The listing builds one solid part. Answer for the finished solid, in the listing's coordinates (mm). Coordinates: 2 decimals unless noted, no trailing zeros. Loops run counter-clockwise (first coordinate to the right, second up) from the corner with the lowest first, then second, coordinate; pieces in that order, holes last. Notation, with made-up numbers: (-4.75, 44) - (6.25, 44) arc R15 ccw to (6.25, 52) - close; hole circle Ø6 at (-10.5, 56). An arc over 180 degrees is marked (long way). Return JSON: item names as keys, results as strings. Group by question number.
1. Section C-C (z = 3.4) is taken. Write down the section's boundary in (x, y), and give its area (3 significant figures).
2. Section A-A (y = 13.5) is taken. Write down the section's boundary in (x, z).
3. Each of these flat-tipped pins is pushed along its axis until it touches: P1, Ø3, axis at x = -8.5, y = 6, coming from the -Z side; P2, Ø3.5, axis at x = 13.5, y = 13.5, coming from the +Z side. Where does it stop, or does it pass through?
4. The mould has two halves that part along Y. Classify faces 1 (the face through (-14.71, -11.603, 1.972)), 2 (the face through (0, -16.5, 2)), 3 (the face through (-14.71, 15.397, 1.972)), 4 (the face through (0, 16.5, 2)): pulls with the +Y half, pulls with the -Y half, needs draft (parallel to the pull), parting line crosses it, or undercut.
5. Find the intervals of material crossed by line 1 along Y through (x, z) = (-13.5, 0.95); line 2 along Y through (x, z) = (-12.5, 2.6); line 3 along X through (y, z) = (-13, 1.35), in increasing order.
6. Section B-B (x = -13.5) is taken. Write down the section's boundary in (y, z), and give its area (3 significant figures).
```python
from build123d import *

# Parameters (mm, degrees)
SKETCH1_W                = 35
SKETCH1_H                = 33
BOSS_EXTRUDE1_DEPTH      = 4
M4_CLEARANCE_HOLE1_D     = 4.5
M4_CLEARANCE_HOLE1_DEPTH = 15
M4_CLEARANCE_HOLE1_TIP   = 1.351936393


with BuildPart() as part:
    # Sketch1 → Boss-Extrude1 (new body)
    with BuildSketch(Plane.XY):
        Rectangle(SKETCH1_W, SKETCH1_H)
    extrude(amount=BOSS_EXTRUDE1_DEPTH)

    # M4 Clearance Hole1
    with Locations(Plane.XY.offset(4)):
        with Locations((13.5, 13.5), (-13.5, 13.5), (-13.5, -13.5), (13.5, -13.5)):
            Hole(M4_CLEARANCE_HOLE1_D / 2, depth=M4_CLEARANCE_HOLE1_DEPTH)
            with Locations((0, 0, -(M4_CLEARANCE_HOLE1_DEPTH + M4_CLEARANCE_HOLE1_TIP / 2))):  # 118° drill point
                Cone(0, M4_CLEARANCE_HOLE1_D / 2, M4_CLEARANCE_HOLE1_TIP, mode=Mode.SUBTRACT)


solid = part.part
```
The answers:
{
 "1": {"outline": "(-17.5, -16.5) - (17.5, -16.5) - (17.5, 16.5) - (-17.5, 16.5) - close; hole circle Ø4.5 at (-13.5, -13.5); hole circle Ø4.5 at (-13.5, 13.5); hole circle Ø4.5 at (13.5, -13.5); hole circle Ø4.5 at (13.5, 13.5)", "area": "1,090 mm2"},
 "2": {"outline": "(-17.5, 0) - (-15.75, 0) - (-15.75, 4) - (-17.5, 4) - close; (-11.25, 0) - (11.25, 0) - (11.25, 4) - (-11.25, 4) - close; (15.75, 0) - (17.5, 0) - (17.5, 4) - (15.75, 4) - close"},
 "3": {"P1": "stops at z = 0", "P2": "passes through"},
 "4": {"face 1": "undercut", "face 2": "pulls with the -Y half", "face 3": "undercut", "face 4": "pulls with the +Y half"},
 "5": {"line 1": "y = -16.5 to -15.75, -11.25 to 11.25, 15.75 to 16.5", "line 2": "y = -16.5 to -15.52, -11.48 to 11.48, 15.52 to 16.5", "line 3": "x = -17.5 to -15.69, -11.31 to 11.31, 15.69 to 17.5"},
 "6": {"outline": "(-16.5, 0) - (-15.75, 0) - (-15.75, 4) - (-16.5, 4) - close; (-11.25, 0) - (11.25, 0) - (11.25, 4) - (-11.25, 4) - close; (15.75, 0) - (16.5, 0) - (16.5, 4) - (15.75, 4) - close", "area": "96.0 mm2"}
}
